Can you work these out from the model? Positions are in its coordinate system, mm. Face numbers are marked on the shaded views. A direction names the side the tool comes from. Round coordinates to 2 decimals unless told otherwise and drop trailing zeros. Order: outer loops, then holes, each group sorted by start corner. A loop starts at its lowest first (then second) coordinate and runs counter-clockwise, first axis right, second up. Notation, with made-up numbers: (71, 6.5) -> (122, 6.5) arc R33 ccw to (122, 39.5) -> close; hole circle Ø11 at (37.5, 74). An arc over 180 degrees is marked (long way). Use a Markdown table: item, result. Add a question column.
Q1. If we section it at D-D on x = 80: List the corners of the cut face in (y, z) for me, plus the area to 3 significant figures.
Q2. I need wall thicknesses on line 1 along X through (y, z) = (145, 5.25); line 2 along X through (y, z) = (15, 2.5); line 3 along Y through (x, z) = (15, 7.75). Which ranges of each line are inside material? Lowest first, please. Write a range as [from, to].
Q3. If we section it at A-A on x = 365: List the corners of the cut face in (y, z) for me.
Q4. If we section it at C-C on y = 275: List the corners of the cut face in (x, z) for me, plus the area to 3 significant figures.
Q5. For the marked faces 1 and 2, which set-ups out of +Z, -Z, +X, -X, +Y, -Y let a thin tool reach every point of the face, with its end or its side?
Q6. If we section it at B-B on y = 145: List the corners of the cut face in (x, z) for me, plus the area to 3 significant figures.
Q7. I'm going to push flat-ended pins straight in: pin 1 Ø0.5 at (x, z) = (203, 11.5) entering from -Y; pin 2 Ø0.5 at (y, z) = (181.5, 11.5) entering from +X. Where does each tip first touch, or does it pass through?
```python
from build123d import *

# Parameters (mm, degrees)
SKETCH1_R           = 7
BOSS_EXTRUDE1_DEPTH = 12
SKETCH2_OUTSIDE_W   = 477.634
SKETCH2_OUTSIDE_H   = 387.634
CUT_EXTRUDE1_DEPTH  = 1


with BuildPart() as part:
    # Sketch1 → Boss-Extrude1 (new body)
    with BuildSketch(Plane.XY):
        with BuildLine():
            Line((10, 0), (370, 0))
            ThreePointArc((370, 0), (377.071067812, 2.928932188), (380, 10))
            Line((380, 10), (380, 280))
            ThreePointArc((380, 280), (377.071067812, 287.071067812), (370, 290))
            Line((370, 290), (10, 290))
            ThreePointArc((10, 290), (2.928932188, 287.071067812), (0, 280))
            Line((0, 280), (0, 10))
            ThreePointArc((0, 10), (2.928932188, 2.928932188), (10, 0))
        make_face()
        with Locations((15, 275)):
            Circle(SKETCH1_R, mode=Mode.SUBTRACT)
        with Locations((131.5, 275)):
            Circle(SKETCH1_R, mode=Mode.SUBTRACT)
        with Locations((248.5, 275)):
            Circle(SKETCH1_R, mode=Mode.SUBTRACT)
        with Locations((365, 275)):
            Circle(SKETCH1_R, mode=Mode.SUBTRACT)
        with Locations((365, 145)):
            Circle(SKETCH1_R, mode=Mode.SUBTRACT)
        with Locations((365, 15)):
            Circle(SKETCH1_R, mode=Mode.SUBTRACT)
        with Locations((248.5, 15)):
            Circle(SKETCH1_R, mode=Mode.SUBTRACT)
        with Locations((131.5, 15)):
            Circle(SKETCH1_R, mode=Mode.SUBTRACT)
        with Locations((15, 15)):
            Circle(SKETCH1_R, mode=Mode.SUBTRACT)
        with Locations((15, 145)):
            Circle(SKETCH1_R, mode=Mode.SUBTRACT)
    extrude(amount=BOSS_EXTRUDE1_DEPTH)

    # Sketch2 outside → Cut-Extrude1 (cut)
    with BuildSketch(Plane.XY.offset(12)):
        with Locations((190, 145)):
            Rectangle(SKETCH2_OUTSIDE_W, SKETCH2_OUTSIDE_H)
        with BuildLine():
            Line((50, 250), (330, 250))
            ThreePointArc((330, 250), (337.071067812, 247.071067812), (340, 240))
            Line((340, 240), (340, 50))
            ThreePointArc((340, 50), (337.071067812, 42.928932188), (330, 40))
            Line((330, 40), (50, 40))
            ThreePointArc((50, 40), (42.928932188, 42.928932188), (40, 50))
            Line((40, 50), (40, 240))
            ThreePointArc((40, 240), (42.928932188, 247.071067812), (50, 250))
        make_face(mode=Mode.SUBTRACT)
    extrude(amount=-CUT_EXTRUDE1_DEPTH, mode=Mode.SUBTRACT)


solid = part.part
```
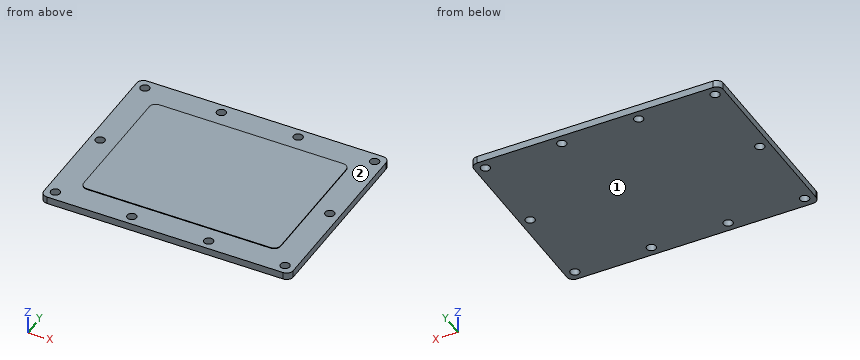
Answer below:
| question | item | result |
|---|---|---|
| 1 | outline | (0, 0) -> (290, 0) -> (290, 11) -> (250, 11) -> (250, 12) -> (40, 12) -> (40, 11) -> (0, 11) -> close |
| 1 | area | 3,400 mm² |
| 2 | line 1 | [0, 8], [22, 358], [372, 380] |
| 2 | line 2 | [0, 8], [22, 124.5], [138.5, 241.5], [255.5, 358], [372, 380] |
| 2 | line 3 | [0, 8], [22, 138], [152, 268], [282, 290] |
| 3 | outline | (0, 0) -> (8, 0) -> (8, 11) -> (0, 11) -> close; (22, 0) -> (138, 0) -> (138, 11) -> (22, 11) -> close; (152, 0) -> (268, 0) -> (268, 11) -> (152, 11) -> close; (282, 0) -> (290, 0) -> (290, 11) -> (282, 11) -> close |
| 4 | outline | (0, 0) -> (8, 0) -> (8, 11) -> (0, 11) -> close; (22, 0) -> (124.5, 0) -> (124.5, 11) -> (22, 11) -> close; (138.5, 0) -> (241.5, 0) -> (241.5, 11) -> (138.5, 11) -> close; (255.5, 0) -> (358, 0) -> (358, 11) -> (255.5, 11) -> close; (372, 0) -> (380, 0) -> (380, 11) -> (372, 11) -> close |
| 4 | area | 3,560 mm² |
| 5 | face 1 | -Z, +X, -X, +Y, -Y |
| 5 | face 2 | +Z |
| 6 | outline | (0, 0) -> (8, 0) -> (8, 11) -> (0, 11) -> close; (22, 0) -> (358, 0) -> (358, 11) -> (340, 11) -> (340, 12) -> (40, 12) -> (40, 11) -> (22, 11) -> close; (372, 0) -> (380, 0) -> (380, 11) -> (372, 11) -> close |
| 6 | area | 4,170 mm² |
| 7 | pin 1 | y = 40 |
| 7 | pin 2 | x = 340 |
